from build123d import *

# Parameters (mm, degrees)
CHAMFER1_SIZE = 25.4


with BuildPart() as part:
    # Sketch1 → Revolve1 (revolve)
    with BuildSketch(Plane.XY, mode=Mode.PRIVATE) as revolve1_sk:
        Polygon((-1244.6, 0), (1244.6, 0), (1244.6, 165.1), (838.2, 165.1), (838.2, 241.3), (-838.2, 241.3), (-838.2, 165.1), (-1244.6, 165.1), align=None)
    revolve(revolve1_sk.sketch.rotate(Axis((-1244.6, 0, 0), (1, 0, 0)), 90), axis=Axis((-1244.6, 0, 0), (1, 0, 0)))

    # Chamfer1
    chamfer1_edges = [part.edges().sort_by_distance(p)[0] for p in [
        (-1244.6, 0, -165.1),
        (1244.6, 0, -165.1),
    ]]
    chamfer(chamfer1_edges, length=CHAMFER1_SIZE)


solid = part.part
Geometry check sheet. Reference: the model listing, model coordinates, mm. A direction names the side the tool comes from. Give positions to 0.01 mm unless a question says otherwise; leave off trailing zeros. Loops run counter-clockwise (first coordinate to the right, second up) from the corner with the lowest first, then second, coordinate; pieces in that order, holes last. Notation, with made-up numbers: M 38.25,-29 L 78.25,-29 A19 ccw 78.25,-8 Z; hole C 58,39.5 d6. An arc over 180 degrees is marked long. Answer as a JSON object with one key per item and string values. Group by question number.
Item 1: Access from +Z, -Z, +X, -X, +Y, -Y to the whole of each face (thin tool, end or side, straight path). Record for faces 1 (the cylindrical face through (1026.033, -163.695, -21.493)), 2 (the cylindrical face through (-1031.367, -163.695, -21.493)), 3 (the cylindrical face through (-11.735, -10.61, -241.067)).
Item 2: Sectioned sample at C-C on x = -1018. Record the boundary of the cut face in (y, z).
Item 3: Sectioned sample at D-D on x = -684.5. Record the boundary of the cut face in (y, z).
Item 4: Gauge pin test, flat ends, axial feed: pin 1 (2 mm diameter, centred on y = 95.5, z = -116.5, fed in from -X); pin 2 (8 mm diameter, centred on x = 803.5, z = 169, fed in from +Y); pin 3 (5 mm diameter, centred on x = -831.5, z = -95, fed in from -Y). Record the tip position at first contact, or that the pin passes through.
Item 5: Sectioned sample at A-A on y = 0. Record the boundary of the cut face in (x, z), plus the area to 3 significant figures.
Item 6: Material ranges on L1, parallel to Z at x = 411, y = -0.5; L2, parallel to X at y = -151, z = -179; L3, parallel to Z at x = -689, y = -7, recorded low to high.
Findings below:
{
 "1": {"face 1": "+X", "face 2": "-X", "face 3": "+X, -X"},
 "2": {"outline": "C 0,0 d330.2"},
 "3": {"outline": "C 0,0 d482.6"},
 "4": {"pin 1": "x = -1234.66", "pin 2": "y = 176.07", "pin 3": "y = -222.87"},
 "5": {"outline": "M -1244.6,-139.7 L -1219.2,-165.1 L -838.2,-165.1 L -838.2,-241.3 L 838.2,-241.3 L 838.2,-165.1 L 1219.2,-165.1 L 1244.6,-139.7 L 1244.6,139.7 L 1219.2,165.1 L 838.2,165.1 L 838.2,241.3 L -838.2,241.3 L -838.2,165.1 L -1219.2,165.1 L -1244.6,139.7 Z", "area": "1,080,000 mm2"},
 "6": {"L1": "-241.3 to 241.3", "L2": "-838.2 to 838.2", "L3": "-241.2 to 241.2"}
}
